Design review of the part built by this model. Coordinates are the model's own, in mm. Face numbers are marked on the shaded views. A direction names the side the tool comes from. Coordinates: 2 decimals unless noted, no trailing zeros. Write each loop counter-clockwise with the first axis right and the second up, starting at its lowest first coordinate (ties: lowest second). Pieces come first, ordered by that corner, then holes.
Q1. For the marked faces 4, 5 and 6, list the 3-axis set-ups (+Z, -Z, +X, -X, +Y, -Y) from which the entire face can be reached by the end or side of a thin tool; tool diameter is ignored.
Q2. For pin 1 Ø1 at (x, y) = (66, 16.5) entering from +Z; pin 2 Ø4 at (x, z) = (103.5, -10.5) entering from +Y; pin 3 Ø6 at (x, z) = (66, 53.5) entering from -Y, all flat-tipped, find the tip position at first contact; note any pin that passes through.
Q3. Take a section at C-C, the plane y = -57.5. Write out the cut boundary in (x, z).
Q4. Take a section at A-A, the plane x = 37.5. Write out the cut boundary in (y, z), plus the area to 3 significant figures.
Q5. Take a section at B-B, the plane z = 29.5. Write out the cut boundary in (x, y), plus the area to 3 significant figures.
Q6. Take a section at D-D, the plane x = 139. Write out the cut boundary in (y, z), plus the area to 3 significant figures.
Q7. For L1, parallel to Y at x = 63, z = 0; L2, parallel to Y at x = 115, z = 0; L3, parallel to Y at x = 148, z = 0, list the stretches that pass through material, from the lowest coordinate up.
Q8. The part is to be moulded in two halves that separate along Y. For the marked faces 1, 2 and 3, say which applies: released by +Y, released by -Y, zero draft, split by the parting line, or undercut.
from build123d import *

# Parameters (mm, degrees)
KEYWAY_PROFILE_6X6_W = 6
KEYWAY_PROFILE_6X6_H = 6
KEYWAY_CUT_6X6_DEPTH = 211


with BuildPart() as part:
    # Pulley Step Profile → Stepped Pulley Body (revolve)
    with BuildSketch(Plane.XY, mode=Mode.PRIVATE) as stepped_pulley_body_sk:
        Polygon((0, 40), (0, 15), (120, 15), (120, 25), (48, 25), (48, 40), (88, 40), (88, 55), (128, 55), (128, 63), (160, 63), (160, 71), (120, 71), (120, 63), (80, 63), (80, 55), (40, 55), (40, 40), align=None)
    revolve(stepped_pulley_body_sk.sketch.rotate(Axis((-51.578947368, 0, 0), (1, 0, 0)), 90), axis=Axis((-51.578947368, 0, 0), (1, 0, 0)))

    # Keyway Profile 6x6 → Keyway Cut 6x6 (cut)
    with BuildSketch(Plane.ZY):
        with Locations((0, 15)):
            Rectangle(KEYWAY_PROFILE_6X6_W, KEYWAY_PROFILE_6X6_H)
    extrude(amount=-KEYWAY_CUT_6X6_DEPTH, mode=Mode.SUBTRACT)


solid = part.part
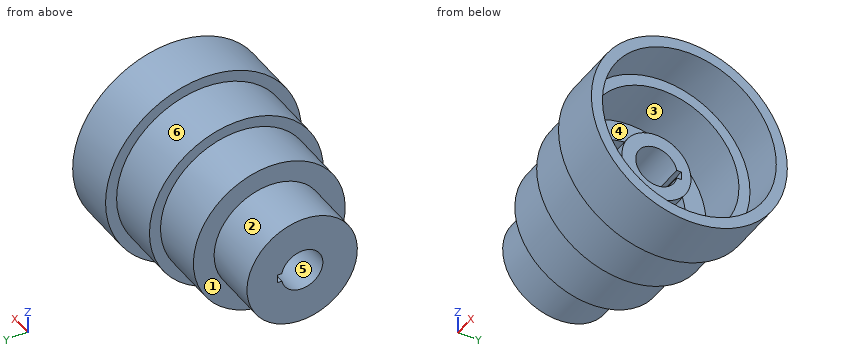
Responses:
1. face 4: +X
1. face 5: +X, -X
1. face 6: -X
2. pin 1: stops at z = 52.62
2. pin 2: stops at y = 62.42
2. pin 3: stops at y = -21.79
3. outline: (80, -25.74) - (120, -25.74) - (120, -41.65) - (160, -41.65) - (160, -25.74) - (128, -25.74) - (128, 25.74) - (160, 25.74) - (160, 41.65) - (120, 41.65) - (120, 25.74) - (80, 25.74) - close
4. outline: circle Ø80 at (0, 0); hole (14.7, -3) - (18, -3) - (18, 3) - (14.7, 3) arc R15 ccw (long way) to start
4. area: 4,300 mm2
5. outline: (0, -27.01) - (40, -27.01) - (40, -46.42) - (80, -46.42) - (80, -55.67) - (120, -55.67) - (120, -64.58) - (160, -64.58) - (160, -55.67) - (128, -55.67) - (128, -46.42) - (88, -46.42) - (88, -27.01) - (48, -27.01) - (48, 27.01) - (88, 27.01) - (88, 46.42) - (128, 46.42) - (128, 55.67) - (160, 55.67) - (160, 64.58) - (120, 64.58) - (120, 55.67) - (80, 55.67) - (80, 46.42) - (40, 46.42) - (40, 27.01) - (0, 27.01) - close
5. area: 6,060 mm2
6. outline: circle Ø142 at (0, 0); hole circle Ø126 at (0, 0)
6. area: 3,370 mm2
7. L1: y = -55 to -40, -25 to -15, 18 to 25, 40 to 55
7. L2: y = -63 to -55, -25 to -15, 18 to 25, 55 to 63
7. L3: y = -71 to -63, 63 to 71
8. face 1: zero draft
8. face 2: split by the parting line
8. face 3: undercut
